Can you work these out from the drawing? Everything is in mm from the part's minimum corner. Round coordinates to 2 decimals unless told otherwise and drop trailing zeros. Loops run counter-clockwise (first coordinate to the right, second up) from the corner with the lowest first, then second, coordinate; pieces in that order, holes last. Notation, with made-up numbers: (47, -25.5) - (84, -25.5) arc R14 ccw to (84, -20.5) - close; hole circle Ø6 at (12, 40). An arc over 180 degrees is marked (long way). Put each result on its own line as item: value. Start each with the question number.
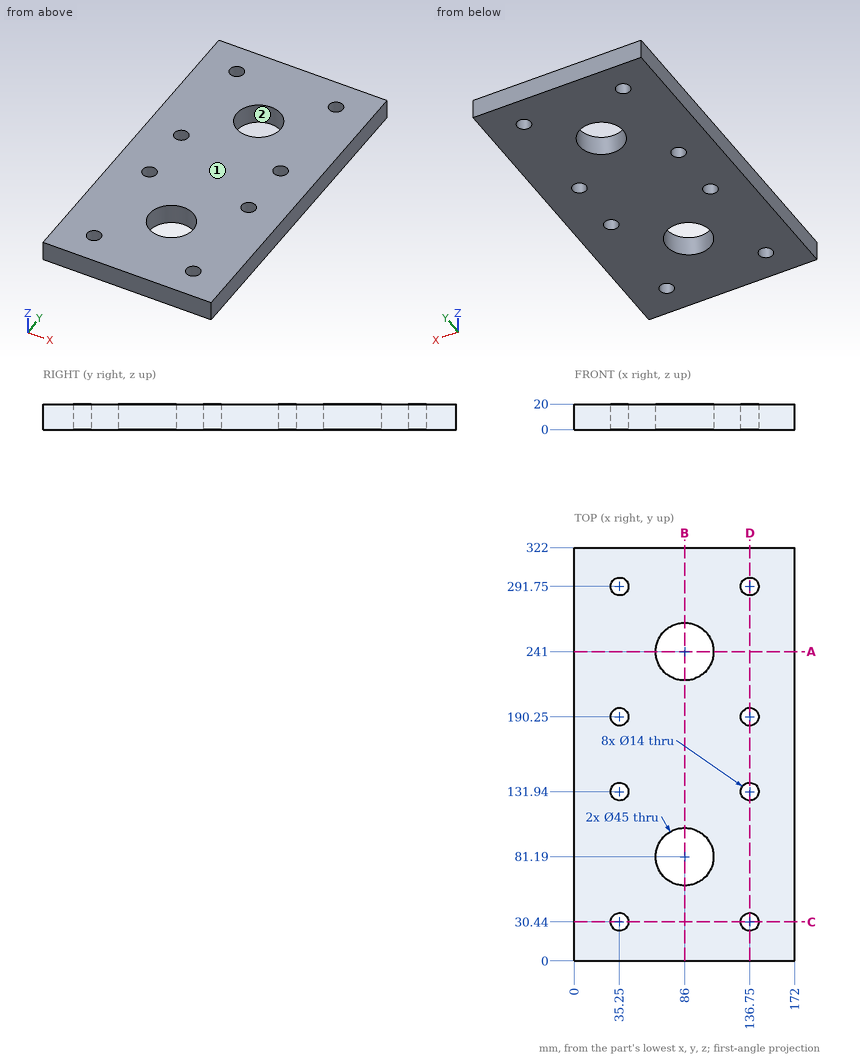
Item 1: Suppose I cut it at B-B, the plane x = 86. List the corners of the cut face in (y, z) for me, then the cut area to 3 significant figures.
Item 2: I need wall thicknesses on line 1 (Y direction, x = 136, z = 5); line 2 (Y direction, x = 35.25, z = 5.5); line 3 (Y direction, x = 70, z = 6.75). Which ranges of each line are inside material? Lowest first, please. Write a range as from..to.
Item 3: Will this pin go through, and if not, where does the flat tip stop? P1, Ø4, axis at x = 97, y = 204.5, coming from the -Z side.
Item 4: Suppose I cut it at A-A, the plane y = 241. List the corners of the cut face in (x, z) for me, then the cut area to 3 significant figures.
Item 5: Suppose I cut it at C-C, the plane y = 30.44. List the corners of the cut face in (x, z) for me.
Item 6: Suppose I cut it at D-D, the plane x = 136.75. List the corners of the cut face in (y, z) for me, then the cut area to 3 significant figures.
Item 7: Thinking about a two-plate mould opening in X: for the marked faces 1 and 2, which applies, released by +X, released by -X, zero draft, split by the parting line, or undercut?
Numbers:
1. outline: (0, 0) - (58.69, 0) - (58.69, 20) - (0, 20) - close; (103.69, 0) - (218.5, 0) - (218.5, 20) - (103.69, 20) - close; (263.5, 0) - (322, 0) - (322, 20) - (263.5, 20) - close
1. area: 4,640 mm^2
2. line 1: 0..23.48, 37.4..124.98, 138.9..183.29, 197.21..284.79, 298.71..322
2. line 2: 0..23.44, 37.44..124.94, 138.94..183.25, 197.25..284.75, 298.75..322
2. line 3: 0..65.37, 97.01..225.18, 256.82..322
3. P1: z = 0
4. outline: (0, 0) - (63.5, 0) - (63.5, 20) - (0, 20) - close; (108.5, 0) - (172, 0) - (172, 20) - (108.5, 20) - close
4. area: 2,540 mm^2
5. outline: (0, 0) - (28.25, 0) - (28.25, 20) - (0, 20) - close; (42.25, 0) - (129.75, 0) - (129.75, 20) - (42.25, 20) - close; (143.75, 0) - (172, 0) - (172, 20) - (143.75, 20) - close
6. outline: (0, 0) - (23.44, 0) - (23.44, 20) - (0, 20) - close; (37.44, 0) - (124.94, 0) - (124.94, 20) - (37.44, 20) - close; (138.94, 0) - (183.25, 0) - (183.25, 20) - (138.94, 20) - close; (197.25, 0) - (284.75, 0) - (284.75, 20) - (197.25, 20) - close; (298.75, 0) - (322, 0) - (322, 20) - (298.75, 20) - close
6. area: 5,320 mm^2
7. face 1: zero draft
7. face 2: undercut
